from build123d import *

# Parameters (mm, degrees)
CUT_EXTRUDE_START   = 2
SKETCH_2_R          = 11
CUT_EXTRUDE_1_DEPTH = 24.323580908
CUT_EXTRUDE_START_2 = 6
SKETCH_3_R          = 11.75
CUT_EXTRUDE_2_DEPTH = 1.1
CHAMFER_1_SIZE      = 0.5


with BuildPart() as part:
    # 草图1 → 旋转1 (revolve)
    with BuildSketch(Plane.XY, mode=Mode.PRIVATE) as revolve_1_sk:
        Polygon((0, 9.5), (0, 13), (2.85, 13), (2.85, 15.825), (7.15, 15.825), (7.15, 13), (11.85, 13), (11.85, 9.5), align=None)
    revolve(revolve_1_sk.sketch.rotate(Axis((0, 0, 0), (1, 0, 0)), 90), axis=Axis((0, 0, 0), (1, 0, 0)))

    # 草图2 → 切除-拉伸1 (cut, through all)
    with BuildSketch(Plane(origin=(0, 0, 0), x_dir=(0, 0, -1), z_dir=(1, 0, 0)).offset(CUT_EXTRUDE_START)):
        Circle(SKETCH_2_R)
    extrude(amount=CUT_EXTRUDE_1_DEPTH, mode=Mode.SUBTRACT)

    # 草图3 → 切除-拉伸2 (cut)
    with BuildSketch(Plane(origin=(2, 0, 0), x_dir=(0, 0, -1), z_dir=(1, 0, 0)).offset(CUT_EXTRUDE_START_2)):
        Circle(SKETCH_3_R)
    extrude(amount=CUT_EXTRUDE_2_DEPTH, mode=Mode.SUBTRACT)

    # 倒角1
    chamfer_1_edges = [part.edges().sort_by_distance(p)[0] for p in [
        (11.85, 0, -13),
        (0, 0, -13),
    ]]
    chamfer(chamfer_1_edges, length=CHAMFER_1_SIZE)


solid = part.part
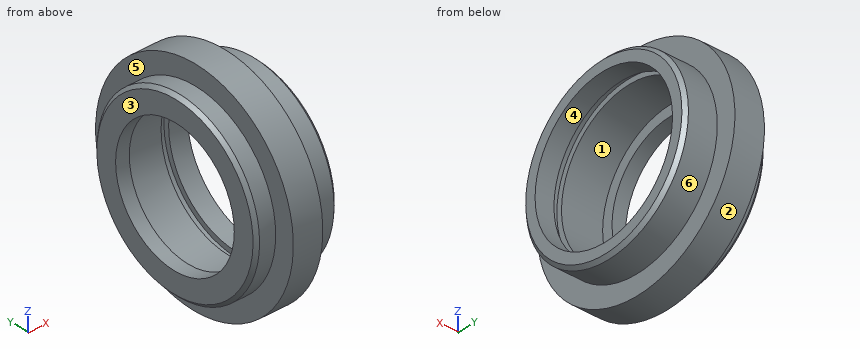
Check sheet for the modelled part. Datum: model origin and axes. Units: mm. Face numbers are marked on the shaded views. A direction names the side the tool comes from. Give positions to 0.01 mm unless a question says otherwise; leave off trailing zeros. Loops run counter-clockwise (first coordinate to the right, second up) from the corner with the lowest first, then second, coordinate; pieces in that order, holes last. Notation, with made-up numbers: M 84,16 L 117,16 A5 cw 117,24 Z; hole C 35,49.25 d10. An arc over 180 degrees is marked long. Return JSON: item names as keys, results as strings. Group by question number.
1. Go/stop test with flat-tipped pins: pin 1 (15 mm diameter, centred on y = 0, z = 0, fed in from -X); pin 2 (1 mm diameter, centred on x = 8, y = -10.5, fed in from +Z); pin 3 (9.5 mm diameter, centred on y = 5, z = 1, fed in from +X). Record where each tip stops, or that it passes through.
2. Cross-section at D-D on x = 1.5. Record the boundary of the cut face in (y, z), plus the area to 3 significant figures.
3. Cross-section at C-C on x = 10.25. Record the boundary of the cut face in (y, z).
4. Thickness scan on L1, parallel to Y at x = 8.6, z = 0; L2, parallel to Y at x = 10.3, z = 0; L3, parallel to X at y = 9.5, z = -6. Record the ranges inside material, lowest first.
5. Tool access check on the marked faces 5 and 6. Record the directions out of +Z, -Z, +X, -X, +Y, -Y that give a thin tool (end or side, any length) a straight path to the whole face; none if there is none.
6. Mould release check, pull along Z, two halves, no side actions. Record for the marked faces 1, 2, 3 and 4: released by +Z, released by -Z, zero draft, split by the parting line, or undercut.
Return value:
{
 "1": {"pin 1": "through", "pin 2": "z = 8.31", "pin 3": "x = 2"},
 "2": {"outline": "C 0,0 d26; hole C 0,0 d19", "area": "247 mm^2"},
 "3": {"outline": "C 0,0 d26; hole C 0,0 d22"},
 "4": {"L1": "-13 to -11.75, 11.75 to 13", "L2": "-13 to -11, 11 to 13", "L3": "0 to 8, 9.1 to 11.85"},
 "5": {"face 5": "-X", "face 6": "+X"},
 "6": {"face 1": "undercut", "face 2": "split by the parting line", "face 3": "zero draft", "face 4": "undercut"}
}
